Geometry: final body of the model. Coordinates: model frame, mm. Round coordinates to 2 decimals unless told otherwise and drop trailing zeros. Loops run counter-clockwise (first coordinate to the right, second up) from the corner with the lowest first, then second, coordinate; pieces in that order, holes last. Notation, with made-up numbers: (19.5, 24.25) - (68.5, 24.25) arc R21 cw to (68.5, 45.25) - close; hole circle Ø3 at (-19.5, 71). An arc over 180 degrees is marked (long way). Answer as CSV lines item,"result".
from build123d import *

# Parameters (mm, degrees)
TOOTH_PROFILE_R         = 1
TOOTH_DEPTH             = 20
TOOTH_PATTERN_30X_COUNT = 30


with BuildPart() as part:
    # Pulley Body Profile → Pulley Body (revolve)
    with BuildSketch(Plane.XY, mode=Mode.PRIVATE) as pulley_body_sk:
        Polygon((8, 40), (8, 0), (18, 0), (23, 5), (23, 10), (18, 10), (18, 30), (23, 30), (23, 35), (18, 40), align=None)
    revolve(pulley_body_sk.sketch.rotate(Axis((0, 32.636363636, 0), (0, -1, 0)), 180), axis=Axis((0, 32.636363636, 0), (0, -1, 0)))

    # Tooth Profile → Tooth (add)
    with BuildSketch(Plane.XZ.offset(-30)):
        with Locations(Location((0, 20.5, 0), (0, 0, 180))):
            Circle(TOOTH_PROFILE_R)
    tooth = extrude(amount=TOOTH_DEPTH)

    # Tooth Pattern 30x: Tooth ×30 about axis
    tooth_pattern_30x_axis = Axis((0, 0, 0), (0, 1, 0))
    for i in range(1, TOOTH_PATTERN_30X_COUNT):
        add(tooth.rotate(tooth_pattern_30x_axis, i * 360 / TOOTH_PATTERN_30X_COUNT))


solid = part.part
(1) Section D-D (y = 34). Output: boundary loops of the cut face in (x, z).
Findings below:
outline,"circle Ø46 at (0, 0); hole circle Ø16 at (0, 0)"
(2) Pin query (flat end, axial travel): P1, Ø3, axis at x = 1.5, y = 9, coming from the +Z side; P2, Ø12, axis at y = 17, z = 12, coming from the +X side; P3, Ø23, axis at x = 3, z = -7, coming from the -Y side; P4, Ø2, axis at y = 15.5, z = 3, coming from the -X side. Return the tip coordinate at first contact, or that it passes through.
Findings below:
P1,"z = 23"
P2,"x = 20.5"
P3,"y = 0"
P4,"x = -21.39"
(3) Draft query along X for faces 1 (the face through (2.994, 7.535, -22.804)), 2 (the face through (4, 0, 8)), 3 (the face through (1.73, 19.72, 7.81)). Return one class per face: pulls with the +X half, pulls with the -X half, needs draft (parallel to the pull), parting line crosses it, or undercut.
Findings below:
face 1,"parting line crosses it"
face 2,"needs draft"
face 3,"undercut"
(4) Section B-B (z = 0). Output: boundary loops of the cut face in (x, y), and give its area (3 significant figures).
Findings below:
outline,"(-23, 5) - (-18, 0) - (-8, 0) - (-8, 40) - (-18, 40) - (-23, 35) - (-23, 30) - (-18, 30) - (-18, 10) - (-23, 10) - close; (8, 0) - (18, 0) - (23, 5) - (23, 10) - (18, 10) - (18, 30) - (23, 30) - (23, 35) - (18, 40) - (8, 40) - close"
area,"950 mm2"
(5) Section C-C (y = 20). Give the number of separate pieces and of enclosed holes in the cut face, and give its area (3 significant figures).
Findings below:
separate pieces,"31"
enclosed holes,"1"
area,"911 mm2"
(6) Section A-A (x = 0). Output: boundary loops of the cut face in (y, z), and give its area (3 significant figures).
Findings below:
outline,"(0, -18) - (5, -23) - (10, -23) - (10, -21.5) - (30, -21.5) - (30, -23) - (35, -23) - (40, -18) - (40, -8) - (0, -8) - close; (0, 8) - (40, 8) - (40, 18) - (35, 23) - (30, 23) - (30, 21.5) - (10, 21.5) - (10, 23) - (5, 23) - (0, 18) - close; hole (10, -19.5) - (30, -19.5) - (30, -18) - (10, -18) - close; hole (10, 18) - (30, 18) - (30, 19.5) - (10, 19.5) - close"
area,"1,030 mm2"
(7) Material intervals for line 1 along Z through (x, y) = (0, 20); line 2 along Z through (x, y) = (-20, 14); line 3 along X through (y, z) = (25, 16.5), sorted ascending.
Findings below:
line 1,"-21.5 to -19.5, -18 to -8, 8 to 18, 19.5 to 21.5"
line 2,"-7.2 to -5.47, -3.06 to -1.22, 1.22 to 3.06, 5.47 to 7.2"
line 3,"-13.05 to -11.05, -7.19 to 7.19, 11.05 to 13.05"
